```python
from build123d import *

# Parameters (mm, degrees)
CHAMFER1_SIZE      = 1.5
CUT_EXTRUDE1_START = -33
CUT_EXTRUDE1_DEPTH = 71
CIRPATTERN1_COUNT  = 6
CHAMFER3_SIZE      = 3.5


with BuildPart() as part:
    # Sketch1 → Revolve1 (revolve)
    with BuildSketch(Plane.XY, mode=Mode.PRIVATE) as revolve1_sk:
        Polygon((-34.5, 28), (-36, 26.5), (-38, 26.5), (-38, 28), (-38, 32.5), (-146, 32.5), (-146, 44.5), (-164, 44.5), (-164, 32.5), (-176, 32.5), (-176, 31.5), (-186, 31.5), (-186, 0), (-176, 0), (-164, 0), (-146, 0), (-38, 0), (0, 0), (0, 28), align=None)
    revolve(revolve1_sk.sketch.rotate(Axis((0, 0, 0), (-1, 0, 0)), 90), axis=Axis((0, 0, 0), (-1, 0, 0)))

    # Chamfer1
    chamfer1_edges = [part.edges().sort_by_distance(p)[0] for p in [
        (0, 0, 28),
    ]]
    chamfer(chamfer1_edges, length=CHAMFER1_SIZE)

    # Sketch2 → Cut-Extrude1 (cut)
    with BuildSketch(Plane(origin=(-38, 0, 0), x_dir=(0, 0, -1), z_dir=(1, 0, 0)).offset(CUT_EXTRUDE1_START)):
        with BuildLine():
            Line((1.79419424, 32.450437085), (27.20580576, 17.779036334))
            ThreePointArc((27.20580576, 17.779036334), (16.25, 28.145825623), (1.79419424, 32.450437085))
        make_face()
    cut_extrude1 = extrude(amount=CUT_EXTRUDE1_DEPTH, mode=Mode.SUBTRACT)

    # CirPattern1: Cut-Extrude1 ×6 about axis
    cirpattern1_axis = Axis((0, 0, 0), (1, 0, 0))
    for i in range(1, CIRPATTERN1_COUNT):
        add(cut_extrude1.rotate(cirpattern1_axis, i * 360 / CIRPATTERN1_COUNT), mode=Mode.SUBTRACT)

    # Sketch4 → Cut-Revolve2 (revolve, cut)
    with BuildSketch(Plane.XY):
        Polygon((0, 0), (-70, 0), (-186, 0), (-186, 21), (-70, 21), (-66.5, 17.5), (0, 17.5), align=None)
    revolve(axis=Axis((0, 0, 0), (-1, 0, 0)), mode=Mode.SUBTRACT)

    # Chamfer3
    chamfer3_edges = [part.edges().sort_by_distance(p)[0] for p in [
        (0, -17.5, 0),
    ]]
    chamfer(chamfer3_edges, length=CHAMFER3_SIZE)


solid = part.part
```
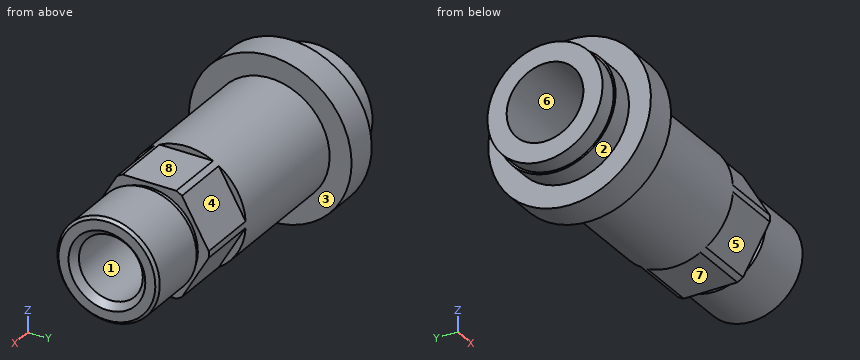
For this review, take the finished solid that the model builds, in its own axes (mm). Face numbers are marked on the shaded views. A direction names the side the tool comes from. Round coordinates to 2 decimals unless told otherwise and drop trailing zeros. Write each loop counter-clockwise with the first axis right and the second up, starting at its lowest first coordinate (ties: lowest second). Pieces come first, ordered by that corner, then holes. Notation, with made-up numbers: (-7.5, 6.5) - (36.5, 6.5) arc R20 ccw to (36.5, 18.5) - close; hole circle Ø2 at (88, 77.5). An arc over 180 degrees is marked (long way). Answer as CSV lines item,"result". Start each with the question number.
(1) Add section B-B, the plane x = -143. State the section outline as (y, z) points.
(2) Mouldability with a two-part tool opening along Y and no side actions: class the marked faces 1, 2 and 3 as +Y half, -Y half, draft (parallel to the pull), parting line (faces both ways), or undercut.
(3) Add section C-C, the plane x = -25. State the section outline as (y, z) points.
(4) Add section A-A, the plane x = -58. State the section outline as (y, z) points, plus the area to 3 significant figures.
(5) Machinability: for the marked faces 4, 5, 6, 7 and 8, which of the approach directions +Z, -Z, +X, -X, +Y, -Y give a long, thin tool a straight path to every point of the face, cutting with its end or side? Answer none if there is none.
(6) For pin 1 (8 mm diameter, centred on x = -124, z = 25.5, fed in from +Y); pin 2 (6 mm diameter, centred on x = -147.5, z = 23, fed in from +Y); pin 3 (9 mm diameter, centred on x = -49.5, y = 0, fed in from +Z); pin 4 (4 mm diameter, centred on y = 6.5, z = 12, fed in from +X), all flat-tipped, find the tip position at first contact; note any pin that passes through.
(7) For line 1 (Z direction, x = -38.5, y = 0); line 2 (Y direction, x = -156.5, z = 0); line 3 (Z direction, x = -115.5, y = 0), list the stretches that pass through material, from the lowest coordinate up.
From the geometry:
1,outline,"circle Ø65 at (0, 0); hole circle Ø42 at (0, 0)"
2,face 1,"undercut"
2,face 2,"parting line"
2,face 3,"draft"
3,outline,"circle Ø56 at (0, 0); hole circle Ø35 at (0, 0)"
4,outline,"(-32.45, -1.79) - (-17.78, -27.21) arc R32.5 ccw to (-14.67, -29) - (14.67, -29) arc R32.5 ccw to (17.78, -27.21) - (32.45, -1.79) arc R32.5 ccw to (32.45, 1.79) - (17.78, 27.21) arc R32.5 ccw to (14.67, 29) - (-14.67, 29) arc R32.5 ccw to (-17.78, 27.21) - (-32.45, 1.79) arc R32.5 ccw to start; hole circle Ø35 at (0, 0)"
4,area,"1,940 mm²"
5,face 4,"+Z, +X, +Y"
5,face 5,"-Z, +X, -Y"
5,face 6,"-X"
5,face 7,"-Z, +X, +Y, -Y"
5,face 8,"+Z, +X, +Y, -Y"
6,pin 1,"stops at y = 24.37"
6,pin 2,"stops at y = 39.75"
6,pin 3,"stops at z = 29"
6,pin 4,"passes through"
7,line 1,"z = -29 to -17.5, 17.5 to 29"
7,line 2,"y = -44.5 to -21, 21 to 44.5"
7,line 3,"z = -32.5 to -21, 21 to 32.5"
